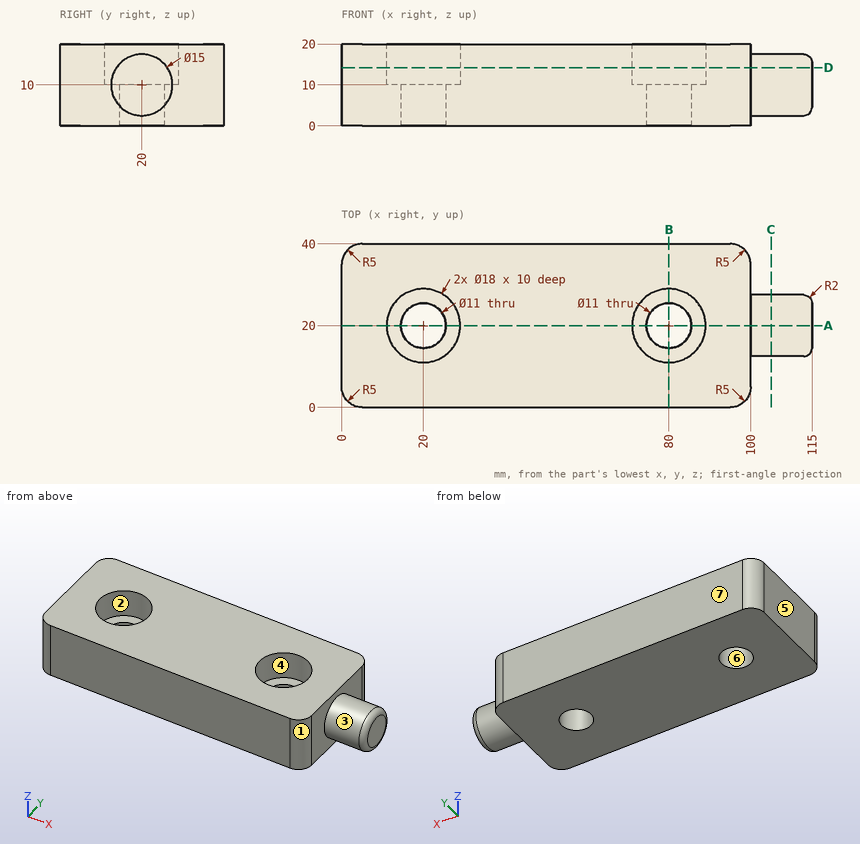
Geometry check sheet. Reference: drawing and pictorial views, mm from the part's lowest x, y, z. A direction names the side the tool comes from. Give positions to 0.01 mm unless a question says otherwise; leave off trailing zeros. Order: outer loops, then holes, each group sorted by start corner. A loop starts at its lowest first (then second) coordinate and runs counter-clockwise, first axis right, second up. Notation, with made-up numbers: M 84,20.25 L 113,20.25 A37 ccw 113,57.25 Z; hole C 13,-36.5 d1. An arc over 180 degrees is marked long. Answer in a Markdown table with one row per item.
1) Cross-section at B-B, the plane x = 80. Enter the section's corners in (y, z), plus the area to 3 significant figures.
Filled sheet:
| item | result |
|---|---|
| outline | M 0,0 L 14.5,0 L 14.5,10 L 11,10 L 11,20 L 0,20 Z; M 25.5,0 L 40,0 L 40,20 L 29,20 L 29,10 L 25.5,10 Z |
| area | 510 mm2 |
2) Gauge pin test, flat ends, axial feed: P1, Ø12.5, axis at x = 80, y = 20, coming from the +Z side; P2, Ø5, axis at y = 9, z = 5, coming from the +X side. Record the tip position at first contact, or that the pin passes through.
Filled sheet:
| item | result |
|---|---|
| P1 | stops at z = 10 |
| P2 | stops at x = 100 |
3) Cross-section at C-C, the plane x = 105. Enter the section's corners in (y, z), plus the area to 3 significant figures.
Filled sheet:
| item | result |
|---|---|
| outline | C 20,10 d15 |
| area | 177 mm2 |
4) Access from +Z, -Z, +X, -X, +Y, -Y to the whole of each face (thin tool, end or side, straight path). Record for the marked faces 1, 2 and 3.
Filled sheet:
| item | result |
|---|---|
| face 1 | +Z, -Z, +X, -Y |
| face 2 | +Z |
| face 3 | +X |
5) Cross-section at D-D, the plane z = 14.25. Count the separate pieces of the cut face and the enclosed holes in it, plus the area to 3 significant figures.
Filled sheet:
| item | result |
|---|---|
| separate pieces | 1 |
| enclosed holes | 2 |
| area | 3,650 mm2 |
6) Release check for a two-part mould opening along Y. For the marked faces 4, 5, 6 and 7 record: +Y half, -Y half, draft (parallel to the pull), parting line (faces both ways), or undercut.
Filled sheet:
| item | result |
|---|---|
| face 4 | undercut |
| face 5 | draft |
| face 6 | undercut |
| face 7 | +Y half |
7) Cross-section at A-A, the plane y = 20. Enter the section's corners in (x, z).
Filled sheet:
| item | result |
|---|---|
| outline | M 0,0 L 14.5,0 L 14.5,10 L 11,10 L 11,20 L 0,20 Z; M 25.5,0 L 74.5,0 L 74.5,10 L 71,10 L 71,20 L 29,20 L 29,10 L 25.5,10 Z; M 85.5,0 L 100,0 L 100,2.5 L 113,2.5 A2 ccw 115,4.5 L 115,15.5 A2 ccw 113,17.5 L 100,17.5 L 100,20 L 89,20 L 89,10 L 85.5,10 Z |
8) Thickness scan on L1, parallel to X at y = 20, z = 5; L2, parallel to Y at x = 20, z = 4.75; L3, parallel to X at y = 20, z = 2. Record the ranges inside material, lowest first. Write a range as [from, to].
Filled sheet:
| item | result |
|---|---|
| L1 | x = [0, 14.5], [25.5, 74.5], [85.5, 115] |
| L2 | y = [0, 14.5], [25.5, 40] |
| L3 | x = [0, 14.5], [25.5, 74.5], [85.5, 100] |
